Input: part model. Units: mm. Frame: model coordinates. A direction names the side the tool comes from. Coordinates: 2 decimals unless noted, no trailing zeros. Loops run counter-clockwise (first coordinate to the right, second up) from the corner with the lowest first, then second, coordinate; pieces in that order, holes last. Notation, with made-up numbers: (-28, 73.5) - (-16, 73.5) arc R8 cw to (-16, 85.5) - close; hole circle Ø6 at (-38, 57.25). An arc over 180 degrees is marked (long way). Use one line per item in the form item = value.
from build123d import *

# Parameters (mm, degrees)
SKETCH1_R           = 9
SKETCH1_R_2         = 2.5
BOSS_EXTRUDE1_DEPTH = 8
SKETCH2_R           = 4.5
CUT_EXTRUDE1_DEPTH  = 5
SKETCH3_R           = 11
CUT_EXTRUDE2_DEPTH  = 7


with BuildPart() as part:
    # Sketch1 → Boss-Extrude1 (new body)
    with BuildSketch(Plane.XY):
        with BuildLine():
            Line((-20, 28.5), (20, 28.5))
            ThreePointArc((20, 28.5), (20.707106781, 28.207106781), (21, 27.5))
            Line((21, 27.5), (21, -28.5))
            Line((21, -28.5), (-21, -28.5))
            Line((-21, -28.5), (-21, 27.5))
            ThreePointArc((-21, 27.5), (-20.707106781, 28.207106781), (-20, 28.5))
        make_face()
        with Locations((0, 14)):
            Circle(SKETCH1_R, mode=Mode.SUBTRACT)
        with Locations((-15, -18.5)):
            Circle(SKETCH1_R_2, mode=Mode.SUBTRACT)
        with Locations((15, -18.5)):
            Circle(SKETCH1_R_2, mode=Mode.SUBTRACT)
    extrude(amount=BOSS_EXTRUDE1_DEPTH)

    # Sketch2 → Cut-Extrude1 (cut)
    with BuildSketch(Plane.XY.offset(8)):
        with Locations((-15, -18.5)):
            Circle(SKETCH2_R)
        with Locations((15, -18.5)):
            Circle(SKETCH2_R)
    extrude(amount=-CUT_EXTRUDE1_DEPTH, mode=Mode.SUBTRACT)

    # Sketch3 → Cut-Extrude2 (cut)
    with BuildSketch(Plane(origin=(0, 0, 0), x_dir=(-1, 0, 0), z_dir=(0, 0, -1))):
        with Locations((0, 14)):
            Circle(SKETCH3_R)
    extrude(amount=-CUT_EXTRUDE2_DEPTH, mode=Mode.SUBTRACT)


solid = part.part
Q1. Pull-direction query (X, two-part tool) for faces 1 (the flat face through (21, 0, 4)), 2 (the flat face through (0, -28.5, 4)), 3 (the flat face through (-13.1, -20.4, 3)); classes: pulls with the +X half, pulls with the -X half, needs draft (parallel to the pull), parting line crosses it, or undercut.
Check values:
face_1 = pulls with the +X half
face_2 = needs draft
face_3 = undercut
Q2. Cut plane A-A, the plane y = 14. Return loops of the section in (x, z).
Check values:
outline = (-21, 0) - (-11, 0) - (-11, 7) - (-9, 7) - (-9, 8) - (-21, 8) - close; (9, 7) - (11, 7) - (11, 0) - (21, 0) - (21, 8) - (9, 8) - close
Q3. Set-up query: faces 4 (the cylindrical face through (12.5, -18.4, 1.5)), 5 (the flat face through (16.9, -20.4, 3)), 6 (the cylindrical face through (2.38, 3.26, 3.45)). Return all of +Z, -Z, +X, -X, +Y, -Y with unobstructed straight access to the full face (end or side cutting, diameter ignored); none if empty.
Check values:
face_4 = +Z, -Z
face_5 = +Z
face_6 = -Z
Q4. Ray query, line 1 along X through (y, z) = (-18.5, 2); line 2 along Y through (x, z) = (15, 1.1); line 3 along Y through (x, z) = (15, 4.6). Return the intervals inside material, ascending. Write a range as [from, to].
Check values:
line_1 = [-21, -17.5], [-12.5, 12.5], [17.5, 21]
line_2 = [-28.5, -21], [-16, 28.5]
line_3 = [-28.5, -23], [-14, 28.5]
Q5. First-contact query: P1, Ø24, axis at x = 1.5, y = 13, coming from the -Z side; P2, Ø20, axis at x = 0, y = 14, coming from the -Z side; P3, Ø3, axis at x = -16.5, y = -21, coming from the +Z side. Flat tips, straight axial feed; report the tip coordinate or a pass-through.
Check values:
P1 = 0
P2 = 7
P3 = 3
Q6. Cut plane B-B, the plane x = -15. Return loops of the section in (y, z).
Check values:
outline = (-28.5, 0) - (-21, 0) - (-21, 3) - (-23, 3) - (-23, 8) - (-28.5, 8) - close; (-16, 0) - (28.5, 0) - (28.5, 8) - (-14, 8) - (-14, 3) - (-16, 3) - close
Q7. Cut plane C-C, the plane z = 4.5. Return loops of the section in (x, y), then the cut area to 3 significant figures.
Check values:
outline = (-21, -28.5) - (21, -28.5) - (21, 27.5) arc R1 ccw to (20, 28.5) - (-20, 28.5) arc R1 ccw to (-21, 27.5) - close; hole circle Ø9 at (-15, -18.5); hole circle Ø22 at (0, 14); hole circle Ø9 at (15, -18.5)
area = 1,890 mm²
